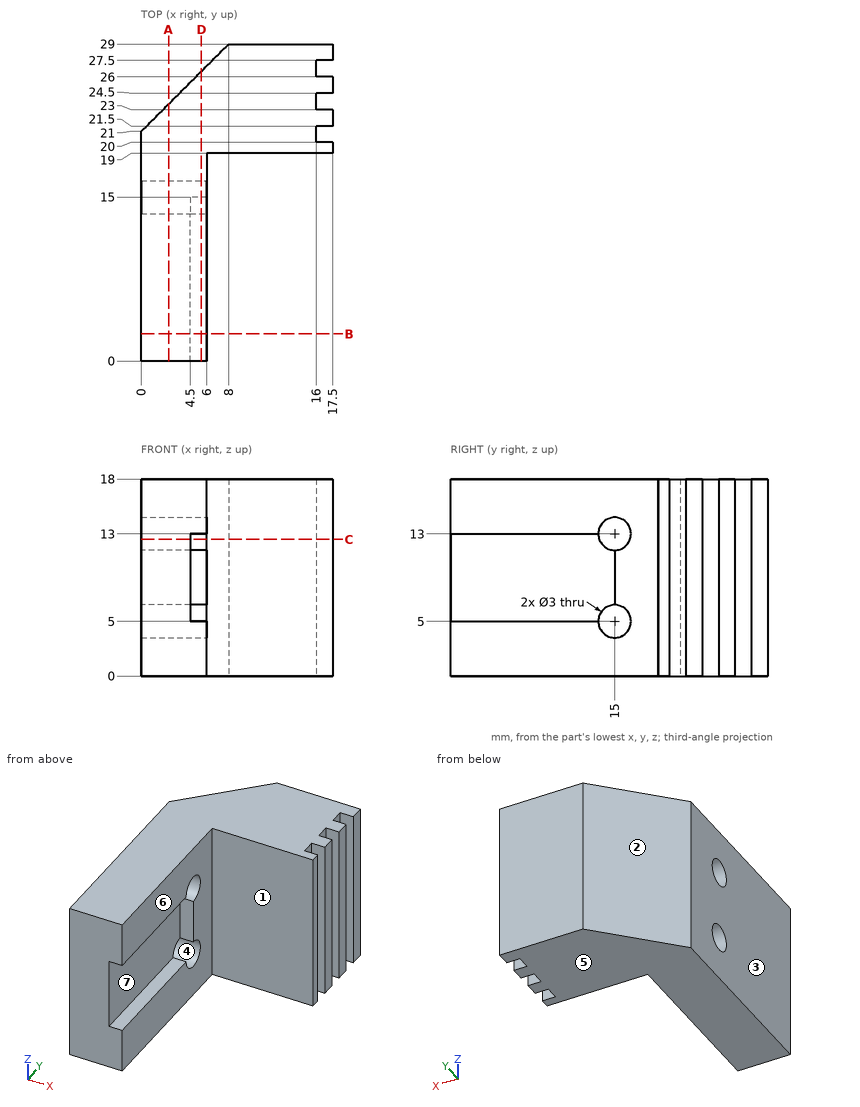
Input: dimensioned drawing with shaded views. Units: mm. Origin: part minimum x, y, z. A direction names the side the tool comes from. Coordinates: 2 decimals unless noted, no trailing zeros. Loops run counter-clockwise (first coordinate to the right, second up) from the corner with the lowest first, then second, coordinate; pieces in that order, holes last. Notation, with made-up numbers: M -24.75,52.5 L 24.25,52.5 A14 ccw 24.25,67.5 Z; hole C 59,-33 d11. An arc over 180 degrees is marked long. Put each result on its own line as item: value.
(1) First-contact query: pin 1 (4 mm diameter, centred on y = 9.5, z = 10.5, fed in from +X); pin 2 (9 mm diameter, centred on x = 14.5, z = 6, fed in from -Y); pin 3 (0.8 mm diameter, centred on x = 5.5, z = 8.5, fed in from -Y). Flat tips, straight axial feed; report the tip coordinate or a pass-through.
Answer sheet:
pin 1: stops at x = 4.5
pin 2: stops at y = 19
pin 3: stops at y = 15
(2) Cut plane A-A on x = 2.5. Return the cut outline in (y, z).
Answer sheet:
outline: M 0,0 L 23.5,0 L 23.5,18 L 0,18 Z; hole C 15,5 d3; hole C 15,13 d3
(3) Cut plane C-C on z = 12.5. Return the cut outline in (x, y).
Answer sheet:
outline: M 0,0 L 4.5,0 L 4.5,13.59 L 0,13.59 Z; M 0,16.41 L 6,16.41 L 6,19 L 17.5,19 L 17.5,20 L 16,20 L 16,21.5 L 17.5,21.5 L 17.5,23 L 16,23 L 16,24.5 L 17.5,24.5 L 17.5,26 L 16,26 L 16,27.5 L 17.5,27.5 L 17.5,29 L 8,29 L 0,21 Z
(4) Material intervals for probe 1 along Z at (x, y) = (3.45, 15); probe 2 along X at (y, z) = (11.25, 15); probe 3 along X at (y, z) = (6.75, 12.5), sorted ascending.
Answer sheet:
probe 1: z = 0 to 3.5, 6.5 to 11.5, 14.5 to 18
probe 2: x = 0 to 6
probe 3: x = 0 to 4.5
(5) Draft query along Y for the marked faces 1, 2, 3 and 4. Return one class per face: pulls with the +Y half, pulls with the -Y half, needs draft (parallel to the pull), parting line crosses it, or undercut.
Answer sheet:
face 1: pulls with the -Y half
face 2: pulls with the +Y half
face 3: needs draft
face 4: undercut
(6) Cut plane D-D on x = 5.5. Return the cut outline in (y, z).
Answer sheet:
outline: M 0,0 L 26.5,0 L 26.5,18 L 0,18 L 0,13 L 13.5,13 A1.5 cw long 15,11.5 L 15,6.5 A1.5 cw long 13.5,5 L 0,5 Z
(7) Access query for the marked faces 5, 6 and 7. Directions: +Z, -Z, +X, -X, +Y, -Y. A direction counts if a zero-diameter tool reaches every point of the face in a straight line with its end or side. Return the directions, or none.
Answer sheet:
face 5: -Z, +X, -X, +Y, -Y
face 6: +Z, -Z, +X, -Y
face 7: +X, -Y
(8) Cut plane B-B on y = 2.5. Return the cut outline in (x, z), then the cut area to 3 significant figures.
Answer sheet:
outline: M 0,0 L 6,0 L 6,5 L 4.5,5 L 4.5,13 L 6,13 L 6,18 L 0,18 Z
area: 96.0 mm^2
